Model file for the job. Use its own axes, mm. A direction names the side the tool comes from. Give positions to 0.01 mm unless a question says otherwise; leave off trailing zeros. Loops run counter-clockwise (first coordinate to the right, second up) from the corner with the lowest first, then second, coordinate; pieces in that order, holes last. Notation, with made-up numbers: M 60,20 L 71,20 A10 ccw 71,32 Z; hole C 48.25,36.5 d8. An arc over 180 degrees is marked long. Use CSV: the item, a comma, the result in double quotes. Start each with the question number.
(1) Slice it at A-A on y = 270. List the corners of the cut face in (x, z).
(2) Slice it at B-B on z = 11.5. List the corners of the cut face in (x, y).
(3) Wall check: line 1 along Y through (x, z) = (0, -55.75); line 2 along Z through (x, y) = (-23.5, 413). Give the ranges that are in metal, low to high. Write a range as from..to.
(4) Two-plate mould, pull along Y, no slides. Class faces 3 (the face through (-20, 483, 50)), 4 (the face through (2.82, 477.31, 54.93)), 5 (the face through (54, 980, 1)): pulls with the +Y half, pulls with the -Y half, needs draft (parallel to the pull), parting line crosses it, or undercut.
(5) Slice it at D-D on y = 580. List the corners of the cut face in (x, z), and give its area (3 significant figures).
(6) Tool access for faces 1 (the face through (-60, 483, -1)), 2 (the face through (20, 483, -50)): list every direction of +Z, -Z, +X, -X, +Y, -Y with a clear straight run to the whole face (end or side of a thin tool).
(7) Slice it at C-C on x = 0. State how many separate pieces and enclosed holes the cut face has, and give its area (3 significant figures).
```python
from build123d import *

# Parameters (mm, degrees)
GB_T6728_2002_120_120_10_1_DEPTH = 980
HOLE_WIZARD_26_1_D               = 26


with BuildPart() as part:
    # Sketch12 → 结构用冷弯空心方钢(gb t6728-2002) 120×120×10(1) (new body)
    with BuildSketch(Plane(origin=(0, 0, 0), x_dir=(-1, 0, 0), z_dir=(0, 1, 0))):
        with BuildLine():
            Line((-44, -60), (44, -60))
            ThreePointArc((44, -60), (55.313708499, -55.313708499), (60, -44))
            Line((60, -44), (60, 44))
            ThreePointArc((60, 44), (55.313708499, 55.313708499), (44, 60))
            Line((44, 60), (-44, 60))
            ThreePointArc((-44, 60), (-55.313708499, 55.313708499), (-60, 44))
            Line((-60, 44), (-60, -44))
            ThreePointArc((-60, -44), (-55.313708499, -55.313708499), (-44, -60))
        make_face()
        with BuildLine():
            Line((-44, -50), (44, -50))
            ThreePointArc((44, -50), (48.242640687, -48.242640687), (50, -44))
            Line((50, -44), (50, 44))
            ThreePointArc((50, 44), (48.242640687, 48.242640687), (44, 50))
            Line((44, 50), (-44, 50))
            ThreePointArc((-44, 50), (-48.242640687, 48.242640687), (-50, 44))
            Line((-50, 44), (-50, -44))
            ThreePointArc((-50, -44), (-48.242640687, -48.242640687), (-44, -50))
        make_face(mode=Mode.SUBTRACT)
    extrude(amount=GB_T6728_2002_120_120_10_1_DEPTH)

    # Ø26 直径孔1 (through all)
    with Locations(Plane.XY.offset(60)):
        with Locations((0, 710), (0, 490), (0, 270)):
            Hole(HOLE_WIZARD_26_1_D / 2)


solid = part.part
```
Reply:
1,outline,"M -60,-44 A16 ccw -44,-60 L -13,-60 L -13,-50 L -44,-50 A6 cw -50,-44 L -50,44 A6 cw -44,50 L -13,50 L -13,60 L -44,60 A16 ccw -60,44 Z; M 13,-60 L 44,-60 A16 ccw 60,-44 L 60,44 A16 ccw 44,60 L 13,60 L 13,50 L 44,50 A6 cw 50,44 L 50,-44 A6 cw 44,-50 L 13,-50 Z"
2,outline,"M -60,0 L -50,0 L -50,980 L -60,980 Z; M 50,0 L 60,0 L 60,980 L 50,980 Z"
3,line 1,"y = 0..257, 283..477, 503..697, 723..980"
3,line 2,"z = -60..-50, 50..60"
4,face 3,"needs draft"
4,face 4,"undercut"
4,face 5,"pulls with the +Y half"
5,outline,"M -60,-44 A16 ccw -44,-60 L 44,-60 A16 ccw 60,-44 L 60,44 A16 ccw 44,60 L -44,60 A16 ccw -60,44 Z; hole M -50,-44 A6 ccw -44,-50 L 44,-50 A6 ccw 50,-44 L 50,44 A6 ccw 44,50 L -44,50 A6 ccw -50,44 Z"
5,area,"4,210 mm^2"
6,face 1,"+Z, -Z, -X, +Y, -Y"
6,face 2,"+Y, -Y"
7,separate pieces,"8"
7,enclosed holes,"0"
7,area,"18,000 mm^2"
